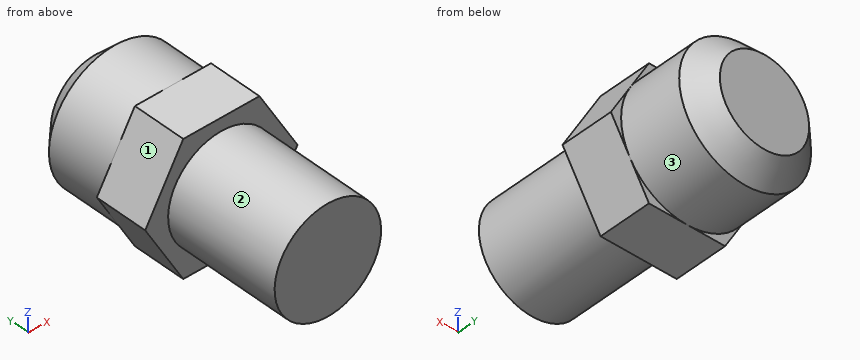
```python
from build123d import *

# Parameters (mm, degrees)
EXTRUDE_1_DEPTH = 5
SKETCH_2_R      = 6.192081637
EXTRUDE_2_DEPTH = 8
CHAMFER_1_SIZE  = 2
SKETCH_3_R      = 5
EXTRUDE_3_DEPTH = 11


with BuildPart() as part:
    # 草图1 → 凸台-拉伸1 (new body)
    with BuildSketch(Plane(origin=(0, 0, 0), x_dir=(1, 0, 0), z_dir=(0, 1, 0))):
        Polygon((-7.15, 0), (-3.575, -6.192081637), (3.575, -6.192081637), (7.15, 0), (3.575, 6.192081637), (-3.575, 6.192081637), align=None)
    extrude(amount=EXTRUDE_1_DEPTH)

    # 草图2 → 凸台-拉伸2 (add)
    with BuildSketch(Plane(origin=(0, 5, 0), x_dir=(1, 0, 0), z_dir=(0, 1, 0))):
        with Locations(Location((0, 0, 0), (0, 0, 270))):
            Circle(SKETCH_2_R)
    extrude(amount=EXTRUDE_2_DEPTH)

    # 倒角1
    chamfer_1_edges = [part.edges().sort_by_distance(p)[0] for p in [
        (0, 13, -6.192081637),
    ]]
    chamfer(chamfer_1_edges, length=CHAMFER_1_SIZE)

    # 草图3 → 凸台-拉伸3 (add)
    with BuildSketch(Plane.XZ):
        with Locations(Location((0, 0, 0), (0, 0, 90))):
            Circle(SKETCH_3_R)
    extrude(amount=EXTRUDE_3_DEPTH)


solid = part.part
```
Could you check a few things on this model? Use its own coordinates, in mm. Face numbers are marked on the shaded views. A direction names the side the tool comes from. Round coordinates to 2 decimals unless told otherwise and drop trailing zeros. Loops run counter-clockwise (first coordinate to the right, second up) from the corner with the lowest first, then second, coordinate; pieces in that order, holes last. Notation, with made-up numbers: M 56,75.5 L 61,75.5 A22 cw 61,101.5 Z; hole C 70,87.25 d7. An arc over 180 degrees is marked long. Write item = value, one per line.
1. I want a section at A-A, the plane y = 7.25. Write out the boundary of the cut face in (x, z).
Results below:
outline = C 0,0 d12.38
2. I need wall thicknesses on probe 1 along X at (y, z) = (-6.75, -3.5); probe 2 along X at (y, z) = (-7.5, -0.25); probe 3 along Y at (x, z) = (-3.75, 5.75). Which ranges of each line are inside material? Lowest first, please.
Results below:
probe_1 = -3.57 to 3.57
probe_2 = -4.99 to 4.99
probe_3 = 0 to 5
3. Will these pins go through, and if not, where does the flat tip stop? P1, Ø3.5, axis at x = 3.5, z = 4, coming from the +Y side; P2, Ø1.4, axis at x = -6, z = 0.5, coming from the +Y side; P3, Ø1, axis at x = 5, y = -2.5, coming from the -Z side; P4, Ø2, axis at x = 4.5, z = 4.5, coming from the +Y side.
Results below:
P1 = 13
P2 = 11.87
P3 = -2.18
P4 = 11.83
4. Which directions (+Z, -Z, +X, -X, +Y, -Y) give clear straight access to the entire face, cutting with the end or side of a thin tool? Please do the marked faces 1, 2 and 3.
Results below:
face_1 = +Z, -X, +Y, -Y
face_2 = -Y
face_3 = +Y
5. I want a section at B-B, the plane y = -4.75. Write out the boundary of the cut face in (x, z).
Results below:
outline = C 0,0 d10
